Build history of the part. All positions in model axes, mm. Face numbers are marked on the shaded views. A direction names the side the tool comes from. Round coordinates to 2 decimals unless told otherwise and drop trailing zeros. Write each loop counter-clockwise with the first axis right and the second up, starting at its lowest first coordinate (ties: lowest second). Pieces come first, ordered by that corner, then holes.
from build123d import *

# Parameters (mm, degrees)
SKETCH1_W           = 80
SKETCH1_H           = 35
SKETCH1_R           = 5.5
SKETCH1_R_2         = 10.5
SKETCH1_W_2         = 15
SKETCH1_H_2         = 50
BOSS_EXTRUDE1_DEPTH = 40
SKETCH2_R           = 6
CUT_EXTRUDE1_DEPTH  = 10
SKETCH4_W           = 50
SKETCH4_H           = 30
CUT_EXTRUDE3_DEPTH  = 81.933614772
SKETCH3_R           = 12.5
CUT_EXTRUDE2_DEPTH  = 15
SKETCH6_W           = 18
SKETCH6_H           = 8
CUT_EXTRUDE4_DEPTH  = 103.46950766
FILLET1_R           = 2
SKETCH7_R           = 2
CUT_EXTRUDE5_DEPTH  = 103.46950766


with BuildPart() as part:
    # Sketch1 → Boss-Extrude1 (new, symmetric)
    # profile 1 of 2: a face of its own
    with BuildSketch(Plane(origin=(0, 0, 0), x_dir=(1, 0, 0), z_dir=(0, 1, 0))):
        with Locations((40, 17.5)):
            Rectangle(SKETCH1_W, SKETCH1_H)
        with Locations(Location((68, 17.5, 0), (0, 0, 270))):
            Circle(SKETCH1_R, mode=Mode.SUBTRACT)
        with Locations(Location((23, 17.5, 0), (0, 0, 270))):
            Circle(SKETCH1_R_2, mode=Mode.SUBTRACT)
    # profile 2 of 2: a face of its own
    with BuildSketch(Plane(origin=(0, 0, 0), x_dir=(1, 0, 0), z_dir=(0, 1, 0))):
        with Locations((23, -25)):
            Rectangle(SKETCH1_W_2, SKETCH1_H_2)
    extrude(amount=BOSS_EXTRUDE1_DEPTH, both=True)

    # Sketch2 → Cut-Extrude1 (cut)
    with BuildSketch(Plane.ZY):
        with Locations((-17.5, 22.5)):
            Circle(SKETCH2_R)
        with Locations((-17.5, -22.5)):
            Circle(SKETCH2_R)
    extrude(amount=-CUT_EXTRUDE1_DEPTH, mode=Mode.SUBTRACT)

    # Sketch4 → Cut-Extrude3 (cut, through all)
    with BuildSketch(Plane(origin=(30.5, 0, 0), x_dir=(0, 0, -1), z_dir=(1, 0, 0))):
        with Locations((-25, -25)):
            Rectangle(SKETCH4_W, SKETCH4_H)
    extrude(amount=-CUT_EXTRUDE3_DEPTH, mode=Mode.SUBTRACT)

    # Sketch3 → Cut-Extrude2 (cut)
    with BuildSketch(Plane(origin=(30.5, 0, 0), x_dir=(0, 0, -1), z_dir=(1, 0, 0))):
        with Locations((-26, 15)):
            Circle(SKETCH3_R)
    extrude(amount=-CUT_EXTRUDE2_DEPTH, mode=Mode.SUBTRACT)

    # Sketch6 → Cut-Extrude4 (cut, through all)
    with BuildSketch(Plane.XY):
        with Locations((71, 0)):
            Rectangle(SKETCH6_W, SKETCH6_H)
    extrude(amount=-CUT_EXTRUDE4_DEPTH, mode=Mode.SUBTRACT)

    # Fillet1
    fillet1_edges = [part.edges().sort_by_distance(p)[0] for p in [
        (55.25, 40, 0),
        (40, -40, 0),
        (0, -40, -17.5),
        (40, -40, -35),
        (80, 40, -17.5),
        (80, -40, -17.5),
        (40, 40, -35),
        (30.5, 15, 50),
        (15.5, 15, 50),
        (15.5, 15, 0),
        (0, 0, 0),
        (0, 0, -35),
        (80, 22, -35),
        (80, 22, 0),
        (30.5, 15, 0),
        (0, 40, -17.5),
        (7.75, 40, 0),
        (15.5, 40, 25),
        (23, 40, 50),
        (15.5, -10, 25),
        (23, -10, 50),
        (23, -10, 0),
        (30.5, -10, 25),
        (30.5, 40, 25),
        (80, -22, 0),
        (80, -22, -35),
    ]]
    fillet(fillet1_edges, radius=FILLET1_R)

    # Sketch7 → Cut-Extrude5 (cut, through all)
    with BuildSketch(Plane.XY):
        with Locations((57, 0)):
            Circle(SKETCH7_R)
    extrude(amount=-CUT_EXTRUDE5_DEPTH, mode=Mode.SUBTRACT)


solid = part.part
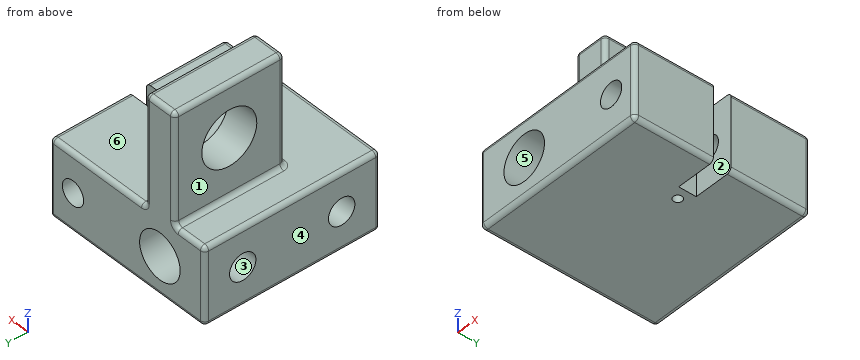
1) Slice it at B-B (y = 15). Write the cut outline in (x, z).
Results:
outline: (0, -33) arc R2 ccw to (2, -35) - (78, -35) arc R2 ccw to (80, -33) - (80, -2) arc R2 ccw to (78, 0) - (32.5, 0) arc R2 cw to (30.5, 2) - (30.5, 13.5) - (15.5, 13.5) - (15.5, 2) arc R2 cw to (13.5, 0) - (2, 0) arc R2 ccw to (0, -2) - close; (15.5, 38.5) - (30.5, 38.5) - (30.5, 48) arc R2 ccw to (28.5, 50) - (17.5, 50) arc R2 ccw to (15.5, 48) - close; hole circle Ø21 at (23, -17.5); hole circle Ø11 at (68, -17.5)
2) Pin check, flat tips, straight feed: pin 1 Ø5 at (x, y) = (71, 8) entering from +Z; pin 2 Ø14 at (y, z) = (7, 22.5) entering from -X; pin 3 Ø12 at (x, z) = (23, 26) entering from -Y; pin 4 Ø12.5 at (x, z) = (23, -17.5) entering from -Y. Stop position of each tip, or through.
Results:
pin 1: stops at z = 0
pin 2: stops at x = 15.5
pin 3: stops at y = -10
pin 4: passes through
3) Slice it at A-A (y = 0). Write the cut outline in (x, z).
Results:
outline: (0, -33) arc R2 ccw to (2, -35) - (55, -35) - (55, 0) - (32.5, 0) arc R2 cw to (30.5, 2) - (30.5, 48) arc R2 ccw to (28.5, 50) - (17.5, 50) arc R2 ccw to (15.5, 48) - (15.5, 2) arc R2 cw to (13.5, 0) - (2, 0) arc R2 ccw to (0, -2) - close; (59, -35) - (62, -35) - (62, 0) - (59, 0) - close; hole circle Ø21 at (23, -17.5)
4) Wall check: L1, parallel to Y at x = 4.5, z = -17.5; L2, parallel to X at y = -11, z = -17.5; L3, parallel to Z at x = 68, y = 26. Give the ranges that are in metal, low to high.
Results:
L1: y = -40 to -28.5, -16.5 to 16.5, 28.5 to 40
L2: x = 0 to 12.5, 33.5 to 62.5, 73.5 to 80
L3: z = -35 to -23, -12 to 0
5) Which spindle directions (+Z, -Z, +X, -X, +Y, -Y) get a long thin tool onto all of the face, cutting with end or side? Do the marked faces 1, 2 and 3. Say none if no direction does.
Results:
face 1: +Z, -X, +Y, -Y
face 2: +Z, -Z, +X
face 3: -X
6) Mould opens along Z. For the marked faces 4, 5 and 6 say: released by +Z, released by -Z, zero draft, split by the parting line, or undercut.
Results:
face 4: zero draft
face 5: undercut
face 6: released by +Z
7) Slice it at C-C (z = -17.5). Count the separate pieces of the cut face and the enclosed holes in it, plus the area to 3 significant figures.
Results:
separate pieces: 4
enclosed holes: 1
area: 3,530 mm2
8) Slice it at D-D (x = 20.5). Write the cut outline in (y, z), plus the area to 3 significant figures.
Results:
outline: (-40, -33) arc R2 ccw to (-38, -35) - (38, -35) arc R2 ccw to (40, -33) - (40, -27.7) - (-40, -27.7) - close; (-40, -7.3) - (40, -7.3) - (40, 48) arc R2 ccw to (38, 50) - (-8, 50) arc R2 ccw to (-10, 48) - (-10, 2) arc R2 cw to (-12, 0) - (-38, 0) arc R2 ccw to (-40, -2) - close; hole circle Ø25 at (15, 26)
area: 3,170 mm2
